The model under review builds one solid part; all positions refer to its coordinate system, in mm. A direction names the side the tool comes from. Give positions to 0.01 mm unless a question says otherwise; leave off trailing zeros. Loops run counter-clockwise (first coordinate to the right, second up) from the corner with the lowest first, then second, coordinate; pieces in that order, holes last. Notation, with made-up numbers: M 50,-10 L 64,-10 A18 cw 64,8 Z; hole C 78.5,56.5 d4. An arc over 180 degrees is marked long. Write item = value, one per line. Start each with the question number.
1. We need section A-A on y = -70. Give the boundary of the cut face in (x, z), then the cut area to 3 significant figures.
2. For faces 5 (the face through (-6, 24, 3)), 6 (the face through (3, -6, 6)), list the 3-axis set-ups (+Z, -Z, +X, -X, +Y, -Y) from which the entire face can be reached by the end or side of a thin tool; tool diameter is ignored.
3. Wall thickness on line 1 along Z through (x, y) = (0, -84); line 2 along Y through (x, z) = (-3, 0); line 3 along X through (y, z) = (81, 150): over which ranges is each line inside the solid? List them lowest first. Write a range as from..to.
4. For pin 1 (9 mm diameter, centred on y = -3, z = -6, fed in from -X); pin 2 (4 mm diameter, centred on x = 0, z = 150, fed in from +Y), all flat-tipped, find the tip position at first contact; note any pin that passes through.
5. Draft analysis for pull direction Z (two halves, no side actions). For faces 1 (the face through (3, -6, -124)), 2 (the face through (0, -100, 3)), 3 (the face through (-1.563, 0.66, -14.985)), 4 (the face through (0, -1, -188)), state which applies: pulls with the +Z half, pulls with the -Z half, needs draft (parallel to the pull), parting line crosses it, or undercut.
from build123d import *

# Parameters (mm, degrees)
SKETCH1_W                  = 376
SKETCH1_H                  = 200
BOSS_EXTRUDE1_DEPTH        = 6
M5_TAPPED_HOLE1_AT_2_COUNT = 2
M5_TAPPED_HOLE1_AT_2_PITCH = 300
M5_TAPPED_HOLE1_AT_3_COUNT = 2
M5_TAPPED_HOLE1_AT_3_PITCH = 150
SKETCH4_R                  = 15
CUT_EXTRUDE1_DEPTH         = 9
SKETCH6_R                  = 8
CUT_EXTRUDE2_DEPTH         = 214.279159788
M4_TAPPED_HOLE1_D          = 3.3
SKETCH9_R                  = 4
CUT_EXTRUDE3_DEPTH         = 214.279159788


with BuildPart() as part:
    # Sketch1 → Boss-Extrude1 (new, symmetric)
    with BuildSketch(Plane(origin=(0, 0, 0), x_dir=(0, 0, -1), z_dir=(1, 0, 0))):
        Rectangle(SKETCH1_W, SKETCH1_H)
    extrude(amount=BOSS_EXTRUDE1_DEPTH, both=True)

    # Sketch3 → M5 Tapped Hole1 (revolve, cut)
    with BuildSketch(Plane(origin=(0, 100, -150), x_dir=(0, 0, 1), z_dir=(1, 0, 0))):
        Polygon((0, 0), (0, 25.7618073), (2.1, 24.5), (2.1, 0), align=None)
    m5_tapped_hole1 = revolve(axis=Axis((0, 106.35, -150), (0, -1, 0)), mode=Mode.SUBTRACT)

    # M5 Tapped Hole1 at 2: M5 Tapped Hole1 ×2
    with Locations(*[(0, 0, i * M5_TAPPED_HOLE1_AT_2_PITCH) for i in range(1, M5_TAPPED_HOLE1_AT_2_COUNT)]):
        add(m5_tapped_hole1, mode=Mode.SUBTRACT)

    # M5 Tapped Hole1 at 3: M5 Tapped Hole1 ×2
    with Locations(*[(0, 0, i * M5_TAPPED_HOLE1_AT_3_PITCH) for i in range(1, M5_TAPPED_HOLE1_AT_3_COUNT)]):
        add(m5_tapped_hole1, mode=Mode.SUBTRACT)

    # Mirror1: M5 Tapped Hole1 across plane
    add(m5_tapped_hole1.mirror(Plane.ZX), mode=Mode.SUBTRACT)

    # Mirror1 copy 1 sketch → Mirror1 copy 1 (revolve, cut)
    with BuildSketch(Plane(origin=(0, -100, 150), x_dir=(0, 0, 1), z_dir=(1, 0, 0))):
        Polygon((0, 0), (0, -25.7618073), (2.1, -24.5), (2.1, 0), align=None)
    revolve(axis=Axis((0, -106.35, 150), (0, -1, 0)), mode=Mode.SUBTRACT)

    # Mirror1 copy 2 sketch → Mirror1 copy 2 (revolve, cut)
    with BuildSketch(Plane(origin=(0, -100, 0), x_dir=(0, 0, 1), z_dir=(1, 0, 0))):
        Polygon((0, 0), (0, -25.7618073), (2.1, -24.5), (2.1, 0), align=None)
    revolve(axis=Axis((0, -106.35, 0), (0, -1, 0)), mode=Mode.SUBTRACT)

    # Sketch4 → Cut-Extrude1 (cut)
    with BuildSketch(Plane.ZY.offset(6)):
        with Locations((-130, 0)):
            Circle(SKETCH4_R)
        Circle(SKETCH4_R)
        with Locations((130, 0)):
            Circle(SKETCH4_R)
    extrude(amount=-CUT_EXTRUDE1_DEPTH, mode=Mode.SUBTRACT)

    # Sketch6 → Cut-Extrude2 (cut, through all)
    with BuildSketch(Plane.ZY.offset(6)):
        with Locations((-130, 0)):
            Circle(SKETCH6_R)
        Circle(SKETCH6_R)
        with Locations((130, 0)):
            Circle(SKETCH6_R)
    extrude(amount=-CUT_EXTRUDE2_DEPTH, mode=Mode.SUBTRACT)

    # M4 Tapped Hole1 (through all)
    with Locations(Plane.ZY.offset(6)):
        with Locations((130, -20), (-150, 0), (-130, 20), (-110, 0), (-130, -20), (-20, 0), (0, 20), (20, 0), (0, -20), (110, 0), (130, 20), (150, 0)):
            Hole(M4_TAPPED_HOLE1_D / 2)

    # Sketch9 → Cut-Extrude3 (cut, through all)
    with BuildSketch(Plane.ZY.offset(6)):
        with Locations((-175, -70)):
            Circle(SKETCH9_R)
        with Locations((-45, -70)):
            Circle(SKETCH9_R)
        with Locations((85, -70)):
            Circle(SKETCH9_R)
    extrude(amount=-CUT_EXTRUDE3_DEPTH, mode=Mode.SUBTRACT)


solid = part.part
Final values:
q1.outline = M -6,-188 L 6,-188 L 6,-179 L -6,-179 Z; M -6,-171 L 6,-171 L 6,-49 L -6,-49 Z; M -6,-41 L 6,-41 L 6,81 L -6,81 Z; M -6,89 L 6,89 L 6,188 L -6,188 Z
q1.area = 4,220 mm²
q2.face_5 = +Z, -Z, -X, +Y, -Y
q2.face_6 = -X
q3.line_1 = -188..-152.1, -147.9..-2.1, 2.1..147.9, 152.1..188
q3.line_2 = -100..-21.65, -18.35..-15, 15..18.35, 21.65..100
q3.line_3 = -6..-2.1, 2.1..6
q4.pin_1 = 3
q4.pin_2 = 75.44
q5.face_1 = undercut
q5.face_2 = needs draft
q5.face_3 = undercut
q5.face_4 = pulls with the -Z half
